```python
from build123d import *

# Parameters (mm, degrees)
BASE_PLATE_5MM_DEPTH           = 5
UPRIGHT_LUG_PROFILE_SKETCH_R   = 3
UPRIGHT_LUG_DEPTH              = 5
PIVOT_START                    = -2.5
PIVOT_COUNTERBORE_SKETCH_R     = 5
PIVOT_COUNTERBORE_SKETCH_R_2   = 3
PIVOT_COUNTERBORE_10X2_5_DEPTH = 2.5


with BuildPart() as part:
    # Base Plate Profile Sketch → Base Plate 5mm (new body)
    with BuildSketch(Plane(origin=(0, 0, 0), x_dir=(1, 0, 0), z_dir=(0, 1, 0))):
        with BuildLine():
            Line((-24, 1), (-24, 0))
            Line((-24, 0), (24, 0))
            Line((24, 0), (24, 1))
            ThreePointArc((24, 1), (23.414213562, 2.414213562), (22, 3))
            Line((22, 3), (16, 3))
            ThreePointArc((16, 3), (11.527864045, 5.763932023), (12, 11))
            ThreePointArc((12, 11), (14.989403432, 20.563724014), (11.290112025, 29.875898463))
            Line((11.290112025, 29.875898463), (4.171208396, 22.756994834))
            ThreePointArc((4.171208396, 22.756994834), (-3.535533906, 16.464466094), (2.756994834, 24.171208396))
            Line((2.756994834, 24.171208396), (10, 31.414213562))
            Line((10, 31.414213562), (10, 35))
            Line((10, 35), (10, 41.180339887))
            Line((10, 41.180339887), (-10, 41.180339887))
            Line((-10, 41.180339887), (-10, 35))
            Line((-10, 35), (-10, 31.180339887))
            ThreePointArc((-10, 31.180339887), (-14.92687273, 21.479348), (-12, 11))
            ThreePointArc((-12, 11), (-11.527864045, 5.763932023), (-16, 3))
            Line((-16, 3), (-22, 3))
            ThreePointArc((-22, 3), (-23.414213562, 2.414213562), (-24, 1))
        make_face()
    extrude(amount=BASE_PLATE_5MM_DEPTH)

    # Upright Lug Profile Sketch → Upright Lug (add)
    with BuildSketch(Plane(origin=(0, 0, -41.180339887), x_dir=(-1, 0, 0), z_dir=(0, 0, -1))):
        with BuildLine():
            Line((-10, 18), (-10, 0))
            Line((-10, 0), (10, 0))
            Line((10, 0), (10, 18))
            ThreePointArc((10, 18), (0, 28), (-10, 18))
        make_face()
        with Locations((0, 18)):
            Circle(UPRIGHT_LUG_PROFILE_SKETCH_R, mode=Mode.SUBTRACT)
    extrude(amount=-UPRIGHT_LUG_DEPTH)

    # Pivot Counterbore Sketch → Pivot Counterbore Ø10x2.5 (cut)
    with BuildSketch(Plane.XY.offset(-36.180339887).offset(PIVOT_START)):
        with Locations((0, 18)):
            Circle(PIVOT_COUNTERBORE_SKETCH_R)
        with Locations(Location((0, 18, 0), (0, 0, 180))):
            Circle(PIVOT_COUNTERBORE_SKETCH_R_2, mode=Mode.SUBTRACT)
    extrude(amount=PIVOT_COUNTERBORE_10X2_5_DEPTH, mode=Mode.SUBTRACT)


solid = part.part
```
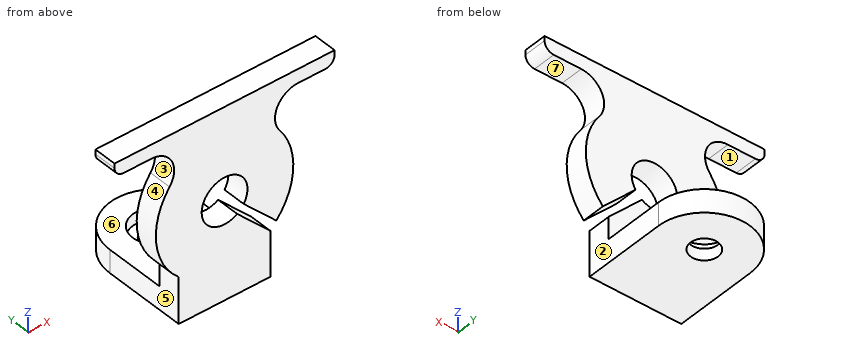
Build history of the part. All positions in model axes, mm. Face numbers are marked on the shaded views. A direction names the side the tool comes from. Round coordinates to 2 decimals unless told otherwise and drop trailing zeros. Order: outer loops, then holes, each group sorted by start corner. A loop starts at its lowest first (then second) coordinate and runs counter-clockwise, first axis right, second up. Notation, with made-up numbers: (2.5, 23) - (50.5, 23) arc R15 ccw to (50.5, 47) - close; hole circle Ø8 at (2.25, 63). An arc over 180 degrees is marked (long way). Use a Markdown table: item, result.
1) Tool access for the marked faces 5, 6 and 7: list every direction of +Z, -Z, +X, -X, +Y, -Y with a clear straight run to the whole face (end or side of a thin tool).
Recorded:
| item | result |
|---|---|
| face 5 | -Z, -X, +Y, -Y |
| face 6 | +Z, +X, -X, +Y |
| face 7 | -Z, +X, +Y, -Y |
2) Pull direction Z, two halves, no side cores. Call the marked faces 1, 2, 3 and 4: pulls with the +Z half, pulls with the -Z half, needs draft (parallel to the pull), parting line crosses it, or undercut.
Recorded:
| item | result |
|---|---|
| face 1 | pulls with the -Z half |
| face 2 | needs draft |
| face 3 | undercut |
| face 4 | undercut |
3) Flat gauge pins, fed straight in: pin 1 Ø11.5 at (x, y) = (0, 18) entering from +Z; pin 2 Ø4 at (x, y) = (18.5, 3.5) entering from -Z; pin 3 Ø10 at (x, y) = (17.5, 17.5) entering from -Z; pin 4 Ø11 at (y, z) = (8.5, -38.5) entering from -X. Where does each tip first touch, or does it go through?
Recorded:
| item | result |
|---|---|
| pin 1 | stops at z = -36.18 |
| pin 2 | stops at z = -3 |
| pin 3 | passes through |
| pin 4 | stops at x = -10 |
4) Saw through at A-A on x = 0. Write the cut outline in (y, z).
Recorded:
| item | result |
|---|---|
| outline | (0, -41.18) - (15, -41.18) - (15, -38.68) - (13, -38.68) - (13, -36.18) - (5, -36.18) - (5, -25) - (0, -25) - close; (0, -15) - (5, -15) - (5, 0) - (0, 0) - close; (21, -41.18) - (28, -41.18) - (28, -36.18) - (23, -36.18) - (23, -38.68) - (21, -38.68) - close |
5) Saw through at D-D on y = 8. Write the cut outline in (x, z), and give its area (3 significant figures).
Recorded:
| item | result |
|---|---|
| outline | (-10, -41.18) - (10, -41.18) - (10, -36.18) - (-10, -36.18) - close |
| area | 100 mm² |
6) Saw through at C-C on x = -13.5. Write the cut outline in (y, z).
Recorded:
| item | result |
|---|---|
| outline | (0, -26.54) - (5, -26.54) - (5, -13.46) - (0, -13.46) - close; (0, -3.67) - (5, -3.67) - (5, 0) - (0, 0) - close |
7) Wall check: L1, parallel to Y at x = 0, z = -36.85; L2, parallel to Z at x = 0, y = 1.7; L3, parallel to X at y = 3.8, z = -20. Give the ranges that are in metal, low to high.
Recorded:
| item | result |
|---|---|
| L1 | y = 0 to 13, 23 to 28 |
| L2 | z = -41.18 to -25, -15 to 0 |
| L3 | x = -15 to -5, 5 to 15 |
8) Saw through at B-B on z = -20. Write the cut outline in (x, y), and give its area (3 significant figures).
Recorded:
| item | result |
|---|---|
| outline | (-15, 0) - (-5, 0) - (-5, 5) - (-15, 5) - close; (5, 0) - (15, 0) - (15, 5) - (5, 5) - close |
| area | 100 mm² |
